Here's how the part is built. I have some questions about the finished solid (model axes, mm). A direction names the side the tool comes from. Round coordinates to 2 decimals unless told otherwise and drop trailing zeros. Loops run counter-clockwise (first coordinate to the right, second up) from the corner with the lowest first, then second, coordinate; pieces in that order, holes last. Notation, with made-up numbers: M -12.75,49 L -5.75,49 A21 cw -5.75,74 Z; hole C 8.5,74.25 d1. An arc over 180 degrees is marked long. Answer as a JSON object with one key per item and string values.
from build123d import *

# Parameters (mm, degrees)
BASE_PLATE_DEPTH        = 5
MOUNTING_HOLES_4_THRU_D = 4
END_LUG_SKETCH_R        = 4
END_LUG_DEPTH           = 10
GUIDE_RAIL_DEPTH        = 17.5


with BuildPart() as part:
    # Base Plate Sketch → Base Plate (new body)
    with BuildSketch(Plane(origin=(0, 0, 0), x_dir=(1, 0, 0), z_dir=(0, 1, 0))):
        with BuildLine():
            Line((-35, -20), (35, -20))
            ThreePointArc((35, -20), (38.535533906, -18.535533906), (40, -15))
            Line((40, -15), (40, 15))
            ThreePointArc((40, 15), (38.535533906, 18.535533906), (35, 20))
            Line((35, 20), (-35, 20))
            ThreePointArc((-35, 20), (-38.535533906, 18.535533906), (-40, 15))
            Line((-40, 15), (-40, -15))
            ThreePointArc((-40, -15), (-38.535533906, -18.535533906), (-35, -20))
        make_face()
    extrude(amount=BASE_PLATE_DEPTH)

    # Mounting Holes Ø4 Thru (through all)
    with Locations(Plane(origin=(-35, 5, -15), x_dir=(0, 0, 1), z_dir=(0, 1, 0))):
        with Locations((0, 0), (0, 70), (30, 70), (30, 0)):
            Hole(MOUNTING_HOLES_4_THRU_D / 2)

    # End Lug Sketch → End Lug (add)
    with BuildSketch(Plane(origin=(40, 0, 0), x_dir=(0, 0, -1), z_dir=(1, 0, 0))):
        with BuildLine():
            Line((-10, 15), (-10, 5))
            Line((-10, 5), (10, 5))
            Line((10, 5), (10, 15))
            ThreePointArc((10, 15), (0, 25), (-10, 15))
        make_face()
        with Locations((0, 15)):
            Circle(END_LUG_SKETCH_R, mode=Mode.SUBTRACT)
    end_lug = extrude(amount=-END_LUG_DEPTH)

    # End Lug Mirror: End Lug across plane
    add(end_lug.mirror(Plane(origin=(0, 0, 0), x_dir=(0, 0, 1), z_dir=(1, 0, 0))))

    # Guide Rail Sketch → Guide Rail (add, symmetric)
    with BuildSketch(Plane(origin=(0, 0, 0), x_dir=(0, 0, -1), z_dir=(1, 0, 0))):
        with BuildLine():
            Line((-20, 5), (-20, 15))
            ThreePointArc((-20, 15), (-15, 20), (-10, 15))
            Line((-10, 15), (-10, 5))
            Line((-10, 5), (-20, 5))
        make_face()
    guide_rail = extrude(amount=GUIDE_RAIL_DEPTH, both=True)

    # Guide Rail Mirror: Guide Rail across plane
    add(guide_rail.mirror(Plane.XY))


solid = part.part
Item 1: I'm going to push flat-ended pins straight in: pin 1 Ø3 at (x, y) = (37, 8.5) entering from +Z; pin 2 Ø3 at (x, y) = (33.5, 10.5) entering from -Z; pin 3 Ø3 at (y, z) = (10.5, -12.5) entering from -X. Where does each tip first touch, or does it pass through?
Resolved:
{"pin 1": "z = 10", "pin 2": "z = -10", "pin 3": "x = -17.5"}
Item 2: I want a section at A-A, the plane y = 7. Please give me the cut outline in (x, z).
Resolved:
{"outline": "M -40,-10 L -30,-10 L -30,10 L -40,10 Z; M -17.5,-20 L 17.5,-20 L 17.5,-10 L -17.5,-10 Z; M -17.5,10 L 17.5,10 L 17.5,20 L -17.5,20 Z; M 30,-10 L 40,-10 L 40,10 L 30,10 Z"}
Item 3: Please list where these lines run through material, in increasing order: probe 1 along X at (y, z) = (2.15, 15); probe 2 along X at (y, z) = (18.75, -5.5); probe 3 along Y at (x, z) = (-34, 0). Write a range as from..to.
Resolved:
{"probe 1": "-40..-37, -33..33, 37..40", "probe 2": "-40..-30, 30..40", "probe 3": "0..11, 19..25"}
Item 4: On a 3-axis mill with a long thin cutter (end or side, diameter ignored), from which of +Z, -Z, +X, -X, +Y, -Y can I reach the whole of each face in a straight line? I mean faces 4 (the face through (17.5, 13, -15)), 5 (the face through (30, 10.7, 0.1)), 6 (the face through (35, 10, -10)), 7 (the face through (-35, 10, -10)). Say none if no direction works.
Resolved:
{"face 4": "+Z, -Z, +X, +Y", "face 5": "+Z, -Z, +Y", "face 6": "-Z, +X, +Y", "face 7": "-Z, -X, +Y"}
Item 5: I want a section at C-C, the plane y = 2.5. Please give me the cut outline in (x, z).
Resolved:
{"outline": "M -40,-15 A5 ccw -35,-20 L 35,-20 A5 ccw 40,-15 L 40,15 A5 ccw 35,20 L -35,20 A5 ccw -40,15 Z; hole C -35,-15 d4; hole C -35,15 d4; hole C 35,-15 d4; hole C 35,15 d4"}
Item 6: If we mould it in two halves opening along Z, with no side actions, what happens to faces 1 (the face through (-37, 2, -15)), 2 (the face through (-38, 2, -19)), 3 (the face through (17.5, 13, 15))? For each: pulls with the +Z half, pulls with the -Z half, needs draft (parallel to the pull), parting line crosses it, or undercut.
Resolved:
{"face 1": "undercut", "face 2": "pulls with the -Z half", "face 3": "needs draft"}
Item 7: I want a section at D-D, the plane x = 2.5. Please give me the cut outline in (y, z).
Resolved:
{"outline": "M 0,-20 L 15,-20 A5 ccw 15,-10 L 5,-10 L 5,10 L 15,10 A5 ccw 15,20 L 0,20 Z"}
Item 8: I want a section at B-B, the plane x = 31. Please give me the cut outline in (y, z), then the cut area to 3 significant figures.
Resolved:
{"outline": "M 0,-20 L 5,-20 L 5,-10 L 15,-10 A10 ccw 15,10 L 5,10 L 5,20 L 0,20 Z; hole C 15,0 d8", "area": "507 mm²"}
